Verification items for this drawing (mm, ordinates from the low corner). A direction names the side the tool comes from. Coordinates: 2 decimals unless noted, no trailing zeros. Loops run counter-clockwise (first coordinate to the right, second up) from the corner with the lowest first, then second, coordinate; pieces in that order, holes last. Notation, with made-up numbers: M 2,71 L 60,71 A22 ccw 60,87 Z; hole C -31.75,43.25 d1. An arc over 180 degrees is marked long. Return JSON: item names as keys, results as strings.
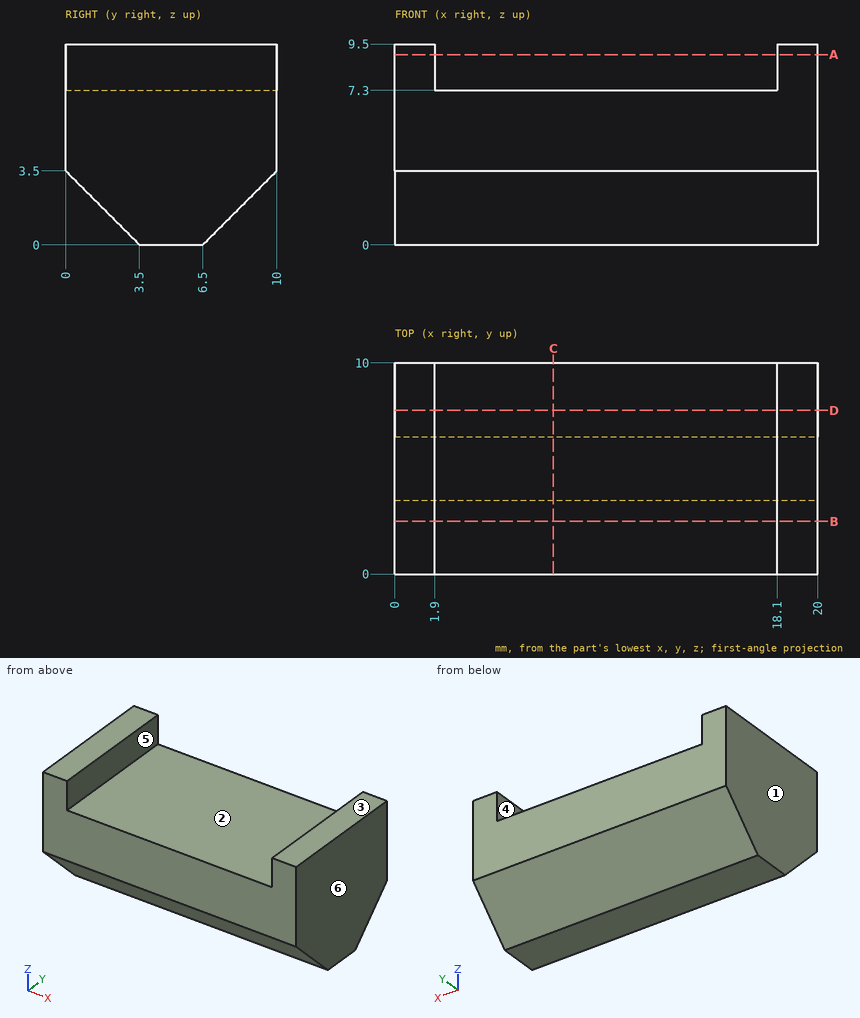
1) Draft check along X on the marked faces 3, 4, 5 and 6. Enter one of: +X half, -X half, draft (parallel to the pull), parting line (faces both ways), or undercut.
Answers:
{"face 3": "draft", "face 4": "undercut", "face 5": "undercut", "face 6": "+X half"}
2) Section check C-C on x = 7.5. Record the cut outline in (y, z).
Answers:
{"outline": "M 0,3.5 L 3.5,0 L 6.5,0 L 10,3.5 L 10,7.3 L 0,7.3 Z"}
3) Go/stop test with a flat-tipped pin: pin 1 Ø3 at (x, y) = (14, 4.5) entering from +Z. Record where the tip stops, or that it passes through.
Answers:
{"pin 1": "z = 7.3"}
4) Set-up check for the marked faces 1 and 2: record each of +Z, -Z, +X, -X, +Y, -Y from which the full face is reachable in a straight line by a thin tool's end or side.
Answers:
{"face 1": "+Z, -Z, -X, +Y, -Y", "face 2": "+Z, +Y, -Y"}
5) Section check B-B on y = 2.5. Record the cut outline in (x, z), then the cut area to 3 significant figures.
Answers:
{"outline": "M 0,1 L 20,1 L 20,9.5 L 18.1,9.5 L 18.1,7.3 L 1.9,7.3 L 1.9,9.5 L 0,9.5 Z", "area": "134 mm²"}
6) Scan lines: line 1 along X through (y, z) = (9.25, 8.25); line 2 along Z through (x, y) = (13.75, 3.75); line 3 along Y through (x, z) = (8, 1.75). Record each from-to range of solid material in increasing order. Write a range as [from, to].
Answers:
{"line 1": "[0, 1.9], [18.1, 20]", "line 2": "[0, 7.3]", "line 3": "[1.75, 8.25]"}
7) Section check A-A on z = 9. Record the cut outline in (x, y).
Answers:
{"outline": "M 0,0 L 1.9,0 L 1.9,10 L 0,10 Z; M 18.1,0 L 20,0 L 20,10 L 18.1,10 Z"}
8) Section check D-D on y = 7.75. Record the cut outline in (x, z).
Answers:
{"outline": "M 0,1.25 L 20,1.25 L 20,9.5 L 18.1,9.5 L 18.1,7.3 L 1.9,7.3 L 1.9,9.5 L 0,9.5 Z"}
